CAD build for the part. Positions are in the model's coordinates, mm. A direction names the side the tool comes from. Coordinates: 2 decimals unless noted, no trailing zeros. Write each loop counter-clockwise with the first axis right and the second up, starting at its lowest first coordinate (ties: lowest second). Pieces come first, ordered by that corner, then holes. Notation, with made-up numbers: M 5.25,68 L 32.25,68 A28 ccw 32.25,98 Z; hole C 47.25,33 d9. An arc over 180 degrees is marked long. Answer as CSV lines item,"result". Start each with the question number.
```python
from build123d import *

# Parameters (mm, degrees)
CHAMFER_1_SIZE      = 1
SKETCH_2_W          = 3.929205492
SKETCH_2_H          = 14.159135618
CUT_EXTRUDE_1_DEPTH = 3.5
CHAMFER_2_SIZE      = 0.5


with BuildPart() as part:
    # 草图1 → 旋转1 (revolve)
    with BuildSketch(Plane.XY, mode=Mode.PRIVATE) as revolve_1_sk:
        Polygon((0, 43), (3.717949192, 43), (5.45, 40), (5.45, 38), (3.45, 36), (3.45, 25), (8.2, 25), (8.2, 20), (6.25, 20), (6.25, 16), (5.2, 16), (5.2, 13.5), (6, 13.5), (6, 0), (0, 0), align=None)
    revolve(revolve_1_sk.sketch.rotate(Axis((0, 0, 0), (0, 1, 0)), 90), axis=Axis((0, 0, 0), (0, 1, 0)))

    # 倒角1
    chamfer_1_edges = [part.edges().sort_by_distance(p)[0] for p in [
        (0, 0, 6),
    ]]
    chamfer(chamfer_1_edges, length=CHAMFER_1_SIZE)

    # 草图2 → 切除-拉伸1 (cut)
    with BuildSketch(Plane(origin=(0, 25, 0), x_dir=(1, 0, 0), z_dir=(0, 1, 0))):
        with Locations((-8.414602746, 0)):
            Rectangle(SKETCH_2_W, SKETCH_2_H)
        with Locations((8.414602746, 0)):
            Rectangle(SKETCH_2_W, SKETCH_2_H)
    extrude(amount=-CUT_EXTRUDE_1_DEPTH, mode=Mode.SUBTRACT)

    # 倒角2
    chamfer_2_edges = [part.edges().sort_by_distance(p)[0] for p in [
        (0, 16, 6.25),
        (0, 20, 8.2),
        (0, 25, 8.2),
        (3.58612191, 25, -7.374261295),
        (-6.45, 25, 0),
        (6.45, 25, 0),
    ]]
    chamfer(chamfer_2_edges, length=CHAMFER_2_SIZE)


solid = part.part
```
1) Probe L1, parallel to Y at x = -1.25, z = 6.5; L2, parallel to X at y = 28.5, z = 0; L3, parallel to Y at x = 6.5, z = -4. List the from-to ranges inside material, lowest first. Write a range as [from, to].
2) Band-saw the part on B-B, the plane y = 38.5. List the corners of the cut face in (x, z).
3) Band-saw the part on C-C, the plane y = 19. List the corners of the cut face in (x, z), plus the area to 3 significant figures.
4) Pin check, flat tips, straight feed: P1, Ø1.5, axis at y = 37.5, z = -4, coming from the -X side; P2, Ø5, axis at x = 5, y = 30, coming from the -Z side; P3, Ø3, axis at y = 10.5, z = -0.5, coming from the +X side. Stop position of each tip, or through.
5) Tool access for faces 5 (the flat face through (-6.3, 20, 1.2)), 6 (the cylindrical face through (4.835, 38.986, -2.515)), 7 (the flat face through (7, 21.5, 0)), 8 (the flat face through (-6.45, 23, 0)), 9 (the flat face through (0, 43, 0)): list every direction of +Z, -Z, +X, -X, +Y, -Y with a clear straight run to the whole face (end or side of a thin tool).
6) Two-plate mould, pull along Y, no slides. Class faces 1 (the flat face through (-7, 21.5, 0)), 2 (the flat face through (4.7, 16, 2.6)), 3 (the cylindrical face through (-5.156, 14.732, 0.677)), 4 (the cylindrical face through (-1.802, 7.162, -5.723)): pulls with the +Y half, pulls with the -Y half, needs draft (parallel to the pull), parting line crosses it, or undercut.
Result sheet:
1,L1,"y = [20, 25]"
1,L2,"x = [-3.45, 3.45]"
1,L3,"y = [20, 21.5]"
2,outline,"C 0,0 d10.9"
3,outline,"C 0,0 d12.5"
3,area,"123 mm²"
4,P1,"stops at x = -4.23"
4,P2,"stops at z = -2.38"
4,P3,"stops at x = 6"
5,face 5,"-Y"
5,face 6,"+Y"
5,face 7,"+Z, -Z, +X, +Y"
5,face 8,"+Z, -Z, -X, +Y"
5,face 9,"+Z, -Z, +X, -X, +Y"
6,face 1,"pulls with the +Y half"
6,face 2,"undercut"
6,face 3,"undercut"
6,face 4,"needs draft"
